Could you check a few things on this model? Use its own coordinates, in mm. Face numbers are marked on the shaded views. A direction names the side the tool comes from. Round coordinates to 2 decimals unless told otherwise and drop trailing zeros. Write each loop counter-clockwise with the first axis right and the second up, starting at its lowest first coordinate (ties: lowest second). Pieces come first, ordered by that corner, then holes. Notation, with made-up numbers: (-11.75, 86.5) -> (31.25, 86.5) arc R30 ccw to (31.25, 124.5) -> close; hole circle Ø5 at (47.5, 60). An arc over 180 degrees is marked (long way). Return JSON: item names as keys, results as strings.
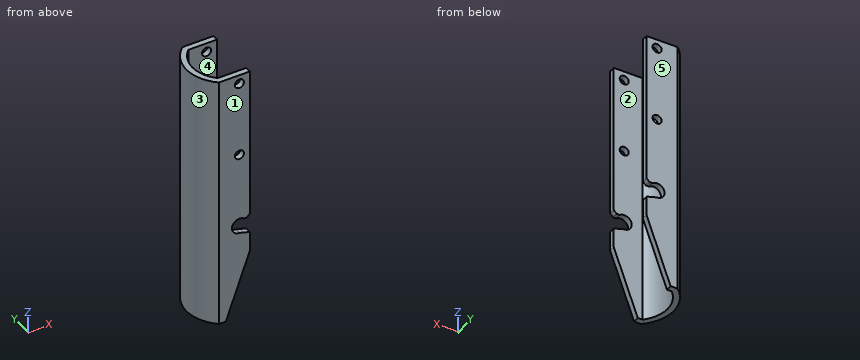
from build123d import *

# Parameters (mm, degrees)
BOSS_EXTRUDE1_DEPTH = 85
SKETCH2_R           = 1.5
CUT_EXTRUDE1_DEPTH  = 89.283633817
CUT_EXTRUDE2_DEPTH  = 89.283633817
FILLET1_R           = 0.5
FILLET2_R           = 0.5


with BuildPart() as part:
    # Sketch1 → Boss-Extrude1 (new body)
    with BuildSketch(Plane.XY):
        with BuildLine():
            Line((-8.306623863, 10), (2, 10))
            Line((2, 10), (2, 8))
            Line((2, 8), (-7.549834435, 8))
            ThreePointArc((-7.549834435, 8), (-11, 0), (-7.549834435, -8))
            Line((-7.549834435, -8), (2, -8))
            Line((2, -8), (2, -10))
            Line((2, -10), (-8.306623863, -10))
            ThreePointArc((-8.306623863, -10), (-13, 0), (-8.306623863, 10))
        make_face()
    extrude(amount=BOSS_EXTRUDE1_DEPTH)

    # Sketch2 → Cut-Extrude1 (cut, through all)
    with BuildSketch(Plane(origin=(0, -10, 0), x_dir=(-1, 0, 0), z_dir=(0, -1, 0))):
        with Locations(Location((1.5, -82, 0), (0, 0, 90))):
            Circle(SKETCH2_R)
        with Locations(Location((1.5, -57, 0), (0, 0, 90))):
            Circle(SKETCH2_R)
        Polygon((-2, -22), (6, 0), (-2, 0), align=None)
    extrude(amount=-CUT_EXTRUDE1_DEPTH, mode=Mode.SUBTRACT)

    # Sketch3 → Cut-Extrude2 (cut, through all)
    with BuildSketch(Plane(origin=(0, -10, 0), x_dir=(-1, 0, 0), z_dir=(0, -1, 0))):
        with BuildLine():
            Line((-2, -28.5), (-2, -35))
            Line((-2, -35), (-1, -34))
            Line((-1, -34), (0, -34))
            ThreePointArc((0, -34), (3.871708245, -32.790569415), (1.5, -29.5))
            Line((1.5, -29.5), (-2, -28.5))
        make_face()
    extrude(amount=-CUT_EXTRUDE2_DEPTH, mode=Mode.SUBTRACT)

    # Fillet1
    fillet1_edges = [part.edges().sort_by_distance(p)[0] for p in [
        (1, -9, 34),
        (1, 9, 34),
        (2, -9, 35),
        (2, 9, 35),
        (0, -9, 34),
        (0, 9, 34),
    ]]
    fillet(fillet1_edges, radius=FILLET1_R)

    # Fillet2
    fillet2_edges = [part.edges().sort_by_distance(p)[0] for p in [
        (-1.5, -9, 29.5),
        (-1.5, 9, 29.5),
    ]]
    fillet(fillet2_edges, radius=FILLET2_R)


solid = part.part
1) I want a section at B-B, the plane z = 32. Please give me the cut outline in (x, y), and give its area (3 significant figures).
Return value:
{"outline": "(-8.31, -10) -> (-4, -10) -> (-4, -8) -> (-7.55, -8) arc R11 cw to (-7.55, 8) -> (-4, 8) -> (-4, 10) -> (-8.31, 10) arc R13 ccw to start", "area": "56.5 mm²"}
2) For the marked faces 1 and 2, which set-ups out of +Z, -Z, +X, -X, +Y, -Y let a thin tool reach every point of the face, with its end or its side?
Return value:
{"face 1": "+Z, -Z, +X, -X, -Y", "face 2": "+Z, -Z, +X"}
3) I want a section at C-C, the plane y = -5.5. Please give me the cut outline in (x, z), and give its area (4 significant figures).
Return value:
{"outline": "(-11.78, 0) -> (-9.53, 0) -> (-9.53, 85) -> (-11.78, 85) -> close", "area": "191.5 mm²"}
4) If I drill on probe 1 along Y at (x, z) = (-6, 34); probe 2 along X at (y, z) = (-9.15, 57); probe 3 along X at (y, z) = (6.75, 36.5), over which ranges is the centre line in solid material (lowest first)? Write a range as [from, to].
Return value:
{"probe 1": "[-10, -8], [8, 10]", "probe 2": "[-9.23, -3], [0, 2]", "probe 3": "[-11.11, -8.69]"}
5) Thinking about a two-plate mould opening in Y: for the marked faces 3, 4 and 5, which applies, pulls with the +Y half, pulls with the -Y half, needs draft (parallel to the pull), parting line crosses it, or undercut?
Return value:
{"face 3": "parting line crosses it", "face 4": "undercut", "face 5": "pulls with the +Y half"}
6) I want a section at D-D, the plane z = 12. Please give me the cut outline in (x, y), and give its area (3 significant figures).
Return value:
{"outline": "(-8.31, -10) -> (-1.64, -10) -> (-1.64, -8) -> (-7.55, -8) arc R11 cw to (-7.55, 8) -> (-1.64, 8) -> (-1.64, 10) -> (-8.31, 10) arc R13 ccw to start", "area": "65.9 mm²"}
7) I want a section at A-A, the plane z = 57. Please give me the cut outline in (x, y).
Return value:
{"outline": "(-8.31, -10) -> (-3, -10) -> (-3, -8) -> (-7.55, -8) arc R11 cw to (-7.55, 8) -> (-3, 8) -> (-3, 10) -> (-8.31, 10) arc R13 ccw to start; (0, -10) -> (2, -10) -> (2, -8) -> (0, -8) -> close; (0, 8) -> (2, 8) -> (2, 10) -> (0, 10) -> close"}
8) Will these pins go through, and if not, where does the flat tip stop? pin 1 Ø2 at (y, z) = (-2, 9) entering from -X; pin 2 Ø5 at (y, z) = (-2.5, 26) entering from +X; pin 3 Ø4 at (y, z) = (5, 18) entering from +X; pin 4 Ø4 at (x, z) = (-1.5, 32) entering from -Y.
Return value:
{"pin 1": "x = -12.96", "pin 2": "x = -9.8", "pin 3": "x = -8.49", "pin 4": "through"}
